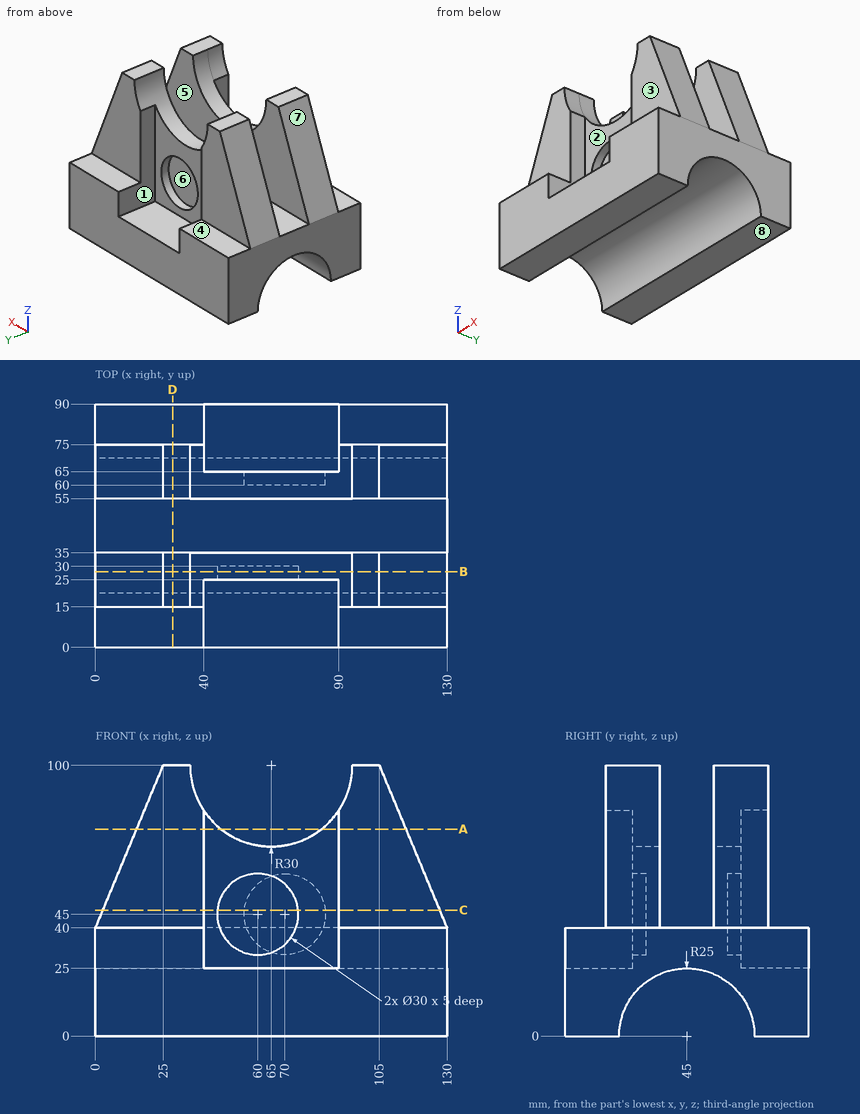
Source: three-view drawing plus pictorial views. Frame: mm from the lowest corner of the part. A direction names the side the tool comes from. Round coordinates to 2 decimals unless told otherwise and drop trailing zeros. Loops run counter-clockwise (first coordinate to the right, second up) from the corner with the lowest first, then second, coordinate; pieces in that order, holes last. Notation, with made-up numbers: M 76,11.5 L 97,11.5 A21 ccw 97,24.5 Z; hole C 31.25,82.25 d11. An arc over 180 degrees is marked long. Answer as CSV lines item,"result". Start each with the question number.
(1) Line query: line 1 (Y direction, x = 32, z = 92); line 2 (Y direction, x = 79, z = 72); line 3 (Z direction, x = 24, y = 13.5). Output: solid intervals per line, ascending. Write a range as [from, to].
(2) Section A-A, the plane z = 76.5. Output: boundary loops of the cut face in (x, y).
(3) Reachability of the marked faces 1, 2, 3, 4 and 5 from +Z, -Z, +X, -X, +Y, -Y: full face, straight path, thin tool, end or side. Return the list, or none.
(4) Section D-D, the plane x = 28.5. Output: boundary loops of the cut face in (y, z).
(5) Section C-C, the plane z = 46.5. Output: boundary loops of the cut face in (x, y), plus the area to 3 significant figures.
(6) Section B-B, the plane y = 28. Output: boundary loops of the cut face in (x, z).
(7) First-contact query: pin 1 (8 mm diameter, centred on x = 104.5, y = 39.5, fed in from -Z); pin 2 (4.5 mm diameter, centred on x = 14, y = 9, fed in from +Z); pin 3 (10 mm diameter, centred on y = 35, z = 52, fed in from +X). Flat tips, straight axial feed; report the tip coordinate or a pass-through.
(8) Draft query along X for the marked faces 6, 7 and 8. Return one class per face: released by +X, released by -X, zero draft, split by the parting line, or undercut.
Values found:
1,line 1,"y = [15, 35], [55, 75]"
1,line 2,"y = [25, 35], [55, 65]"
1,line 3,"z = [0, 40]"
2,outline,"M 15.21,15 L 40,15 L 40,25 L 46.35,25 L 46.35,35 L 15.21,35 Z; M 15.21,55 L 46.35,55 L 46.35,65 L 40,65 L 40,75 L 15.21,75 Z; M 83.65,25 L 90,25 L 90,15 L 114.79,15 L 114.79,35 L 83.65,35 Z; M 83.65,55 L 114.79,55 L 114.79,75 L 90,75 L 90,65 L 83.65,65 Z"
3,face 1,"+Z, +Y"
3,face 2,"+Z, -Y"
3,face 3,"+Z, +X, -X, -Y"
3,face 4,"+Z, +X, -X, +Y"
3,face 5,"+Z, +X, -X"
4,outline,"M 0,0 L 20,0 A25 cw 70,0 L 90,0 L 90,40 L 75,40 L 75,100 L 55,100 L 55,40 L 35,40 L 35,100 L 15,100 L 15,40 L 0,40 Z"
5,outline,"M 2.71,15 L 40,15 L 40,25 L 45.08,25 L 45.08,30 L 74.92,30 L 74.92,25 L 90,25 L 90,15 L 127.29,15 L 127.29,35 L 2.71,35 Z; M 2.71,55 L 127.29,55 L 127.29,75 L 90,75 L 90,65 L 84.92,65 L 84.92,60 L 55.08,60 L 55.08,65 L 40,65 L 40,75 L 2.71,75 Z"
5,area,"3,680 mm²"
6,outline,"M 0,18.33 L 130,18.33 L 130,40 L 105,100 L 95,100 A30 cw 35,100 L 25,100 L 0,40 Z; hole C 60,45 d30"
7,pin 1,"stops at z = 23.12"
7,pin 2,"stops at z = 40"
7,pin 3,"stops at x = 127.08"
8,face 6,"undercut"
8,face 7,"released by -X"
8,face 8,"zero draft"
